Check sheet for the drawn part. Datum: minimum x, y, z corner. Units: mm. Coordinates: 2 decimals unless noted, no trailing zeros. Order: outer loops, then holes, each group sorted by start corner. A loop starts at its lowest first (then second) coordinate and runs counter-clockwise, first axis right, second up. Notation, with made-up numbers: M 18,-10 L 23,-10 A22 ccw 23,6 Z; hole C 11.25,57.5 d6. An arc over 180 degrees is marked long. Return JSON: item names as keys, results as strings. Group by question number.
Q1. Thickness scan on probe 1 along X at (y, z) = (10, 3.2) (1 decimal); probe 2 along X at (y, z) = (11.5, 1.45) (1 decimal); probe 3 along Y at (x, z) = (10.5, 1.6). Record the ranges inside material, lowest first.
Q2. Go/stop test with flat-tipped pins: pin 1 Ø2 at (x, z) = (13, 0.5) entering from +Y; pin 2 Ø1 at (x, z) = (3, 4) entering from +Y; pin 3 Ø2 at (x, z) = (3, 3) entering from -Y; pin 4 Ø1.5 at (y, z) = (4, 4) entering from +X. Record where each tip stops, or that it passes through.
Q3. Mould release check, pull along Y, two halves, no side actions. Record for the marked faces 1, 2 and 3: pulls with the +Y half, pulls with the -Y half, needs draft (parallel to the pull), parting line crosses it, or undercut.
Q4. Section check A-A, the plane z = 2.75. Enter the section's corners in (x, y) (1 decimal), then the cut area to 3 significant figures.
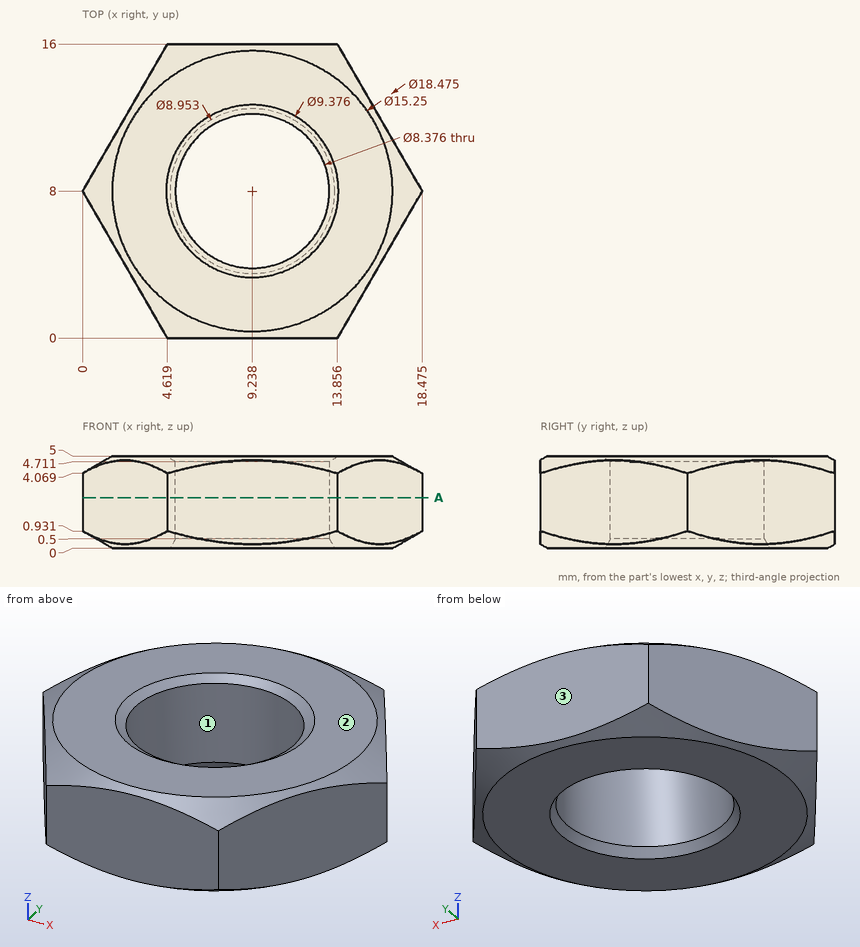
Numbers:
{
 "1": {"probe 1": "x = 1.2 to 5.6, 12.9 to 17.3", "probe 2": "x = 2 to 6.9, 11.5 to 16.5", "probe 3": "y = 0 to 4.01, 11.99 to 16"},
 "2": {"pin 1": "stops at y = 16", "pin 2": "stops at y = 14.06", "pin 3": "stops at y = 1.07", "pin 4": "stops at x = 16.6"},
 "3": {"face 1": "undercut", "face 2": "needs draft", "face 3": "pulls with the +Y half"},
 "4": {"outline": "M 0,8 L 4.6,0 L 13.9,0 L 18.5,8 L 13.9,16 L 4.6,16 Z; hole C 9.2,8 d8.4", "area": "167 mm2"}
}
